Part model, mm, in its own coordinate system. A direction names the side the tool comes from. Round coordinates to 2 decimals unless told otherwise and drop trailing zeros. Loops run counter-clockwise (first coordinate to the right, second up) from the corner with the lowest first, then second, coordinate; pieces in that order, holes last. Notation, with made-up numbers: (-30.75, 12) -> (25.25, 12) arc R13 ccw to (25.25, 31) -> close; hole circle Ø8 at (31, -31.75). An arc over 180 degrees is marked (long way). Answer as CSV lines item,"result".
from build123d import *

# Parameters (mm, degrees)
G1_4_TAPPED_HOLE1_D                               = 11.8
HOLE_SIZE_BASED_ON_SOCKET_HEAD_CAP_SC_D           = 4.8
HOLE_SIZE_BASED_ON_SOCKET_HEAD_CAP_SC_CBORE_D     = 8
HOLE_SIZE_BASED_ON_SOCKET_HEAD_CAP_SC_CBORE_DEPTH = 4.6
FILLET1_R                                         = 0.2
CHAMFER1_SIZE                                     = 0.2
CHAMFER2_SIZE                                     = 0.5
CUT_EXTRUDE1_DEPTH                                = 35.474628352


with BuildPart() as part:
    # Sketch2 → Revolve1 (revolve)
    with BuildSketch(Plane.XY, mode=Mode.PRIVATE) as revolve1_sk:
        Polygon((0, 24), (-17.5, 24), (-17.5, 16), (-7.75, 16), (-7.75, 0), (0, 0), align=None)
    revolve(revolve1_sk.sketch.rotate(Axis((0, 0, 0), (0, 1, 0)), 270), axis=Axis((0, 0, 0), (0, 1, 0)))

    # G1/4 Tapped Hole1 (through all)
    with Locations(Plane.ZX.offset(24)):
        with Locations((0, 0)):
            Hole(G1_4_TAPPED_HOLE1_D / 2)

    # Hole Size (% based on) Socket Head Cap Screw Type 1 (through all)
    with Locations(Plane(origin=(-8.485281374, 24, -8.485281374), x_dir=(0, 0, 1), z_dir=(0, 1, 0))):
        with Locations((0, 0), (16.970562748, 16.970562748)):
            CounterBoreHole(HOLE_SIZE_BASED_ON_SOCKET_HEAD_CAP_SC_D / 2, HOLE_SIZE_BASED_ON_SOCKET_HEAD_CAP_SC_CBORE_D / 2, HOLE_SIZE_BASED_ON_SOCKET_HEAD_CAP_SC_CBORE_DEPTH)

    # Fillet1
    fillet1_edges = [part.edges().sort_by_distance(p)[0] for p in [
        (0, 16, 7.75),
    ]]
    fillet(fillet1_edges, radius=FILLET1_R)

    # Chamfer1
    chamfer1_edges = [part.edges().sort_by_distance(p)[0] for p in [
        (0, 0, 7.75),
        (0, 16, 17.5),
        (0, 24, 17.5),
    ]]
    chamfer(chamfer1_edges, length=CHAMFER1_SIZE)

    # Chamfer2
    chamfer2_edges = [part.edges().sort_by_distance(p)[0] for p in [
        (0, 24, 5.9),
        (0, 0, 5.9),
    ]]
    chamfer(chamfer2_edges, length=CHAMFER2_SIZE)

    # Sketch7 → Cut-Extrude1 (cut, through all)
    with BuildSketch(Plane(origin=(0, 24, 0), x_dir=(1, 0, 0), z_dir=(0, 1, 0))):
        with BuildLine():
            Line((2.911166407, -17.053302031), (-17.053302031, 2.911166407))
            ThreePointArc((-17.053302031, 2.911166407), (-12.232947315, -12.232947315), (2.911166407, -17.053302031))
        make_face()
        with BuildLine():
            ThreePointArc((17.3, 0), (11.156317071, 13.222200627), (-2.911166407, 17.053302031))
            Line((-2.911166407, 17.053302031), (17.053302031, -2.911166407))
            ThreePointArc((17.053302031, -2.911166407), (17.238215179, -1.460800272), (17.3, 0))
        make_face()
        with BuildLine():
            Line((-17.053302031, 2.911166407), (-17.226115818, 3.083980194))
            ThreePointArc((-17.226115818, 3.083980194), (-12.374368671, -12.374368671), (3.083980194, -17.226115818))
            Line((3.083980194, -17.226115818), (2.911166407, -17.053302031))
            ThreePointArc((2.911166407, -17.053302031), (-12.232947315, -12.232947315), (-17.053302031, 2.911166407))
        make_face()
        with BuildLine():
            ThreePointArc((17.5, 0), (11.23121424, 13.42050024), (-3.083980194, 17.226115818))
            Line((-3.083980194, 17.226115818), (-2.911166407, 17.053302031))
            ThreePointArc((-2.911166407, 17.053302031), (11.156317071, 13.222200627), (17.3, 0))
            ThreePointArc((17.3, 0), (17.238215179, -1.460800272), (17.053302031, -2.911166407))
            Line((17.053302031, -2.911166407), (17.226115818, -3.083980194))
            ThreePointArc((17.226115818, -3.083980194), (17.431394477, -1.548058977), (17.5, 0))
        make_face()
    extrude(amount=-CUT_EXTRUDE1_DEPTH, mode=Mode.SUBTRACT)


solid = part.part
Q1. Saw through at B-B, the plane x = 0. Write the cut outline in (y, z), then the cut area to 3 significant figures.
Geometry results:
outline,"(0, -7.55) -> (0.2, -7.75) -> (15.8, -7.75) arc R0.2 cw to (16, -7.95) -> (16, -14.14) -> (24, -14.14) -> (24, -6.4) -> (23.5, -5.9) -> (0.5, -5.9) -> (0, -6.4) -> close; (0, 6.4) -> (0.5, 5.9) -> (23.5, 5.9) -> (24, 6.4) -> (24, 14.14) -> (16, 14.14) -> (16, 7.95) arc R0.2 cw to (15.8, 7.75) -> (0.2, 7.75) -> (0, 7.55) -> close"
area,"191 mm2"
Q2. Which spindle directions (+Z, -Z, +X, -X, +Y, -Y) get a long thin tool onto all of the face, cutting with end or side? Do faces 1 (the face through (9, 19.4, 11)), 2 (the face through (-3, 24, -6)). Say none if no direction does.
Geometry results:
face 1,"+Y"
face 2,"+Z, -Z, +X, -X, +Y"
Q3. Drill centre lines: line 1 along X through (y, z) = (8, 0); line 2 along Z through (x, y) = (-8, 17.5); line 3 along X through (y, z) = (21.75, 1). Where is each one in solid material? Low to high.
Geometry results:
line 1,"-7.75 to -5.9, 5.9 to 7.75"
line 2,"-15.56 to -10.84, -6.13 to 6.14"
line 3,"-13.14 to -5.81, 5.81 to 15.14"
Q4. Saw through at C-C, the plane y = 18.25. Write the cut outline in (x, z), then the cut area to 3 significant figures.
Geometry results:
outline,"(-17.23, -3.08) arc R17.5 ccw to (-3.08, -17.23) -> (17.23, 3.08) arc R17.5 ccw to (3.08, 17.23) -> close; hole circle Ø4.8 at (-8.49, -8.49); hole circle Ø11.8 at (0, 0); hole circle Ø4.8 at (8.49, 8.49)"
area,"514 mm2"
Q5. Drop flat-ended pins along their axis: P1, Ø3, axis at x = 8.49, z = 8.49, coming from the -Y side; P2, Ø3, axis at x = 4.5, z = -10.5, coming from the +Y side; P3, Ø2, axis at y = 16, z = 5, coming from the +X side; P4, Ø6.5, axis at x = 8.49, z = 8.49, coming from the +Y side. Give the stop position or say it passes through.
Geometry results:
P1,"through"
P2,"y = 24"
P3,"x = 17.03"
P4,"y = 19.4"
Q6. Saw through at A-A, the plane z = 0. Write the cut outline in (x, y), then the cut area to 3 significant figures.
Geometry results:
outline,"(-14.14, 16) -> (-7.95, 16) arc R0.2 cw to (-7.75, 15.8) -> (-7.75, 0.2) -> (-7.55, 0) -> (-6.4, 0) -> (-5.9, 0.5) -> (-5.9, 23.5) -> (-6.4, 24) -> (-14.14, 24) -> close; (5.9, 0.5) -> (6.4, 0) -> (7.55, 0) -> (7.75, 0.2) -> (7.75, 15.8) arc R0.2 cw to (7.95, 16) -> (14.14, 16) -> (14.14, 24) -> (6.4, 24) -> (5.9, 23.5) -> close"
area,"191 mm2"
Q7. Saw through at D-D, the plane y = 3. Write the cut outline in (x, z).
Geometry results:
outline,"circle Ø15.5 at (0, 0); hole circle Ø11.8 at (0, 0)"
Q8. Two-plate mould, pull along X, no slides. Class faces 3 (the face through (-8.4, 19.4, -5.9)), 4 (the face through (-7.684, 7.891, 1.009)), 5 (the face through (-4, 16, 8)), 6 (the face through (12.45, 21.73, 7.96)): pulls with the +X half, pulls with the -X half, needs draft (parallel to the pull), parting line crosses it, or undercut.
Geometry results:
face 3,"undercut"
face 4,"parting line crosses it"
face 5,"needs draft"
face 6,"undercut"
